Check sheet for the modelled part. Datum: model origin and axes. Units: mm. Face numbers are marked on the shaded views. A direction names the side the tool comes from. Coordinates: 2 decimals unless noted, no trailing zeros. Write each loop counter-clockwise with the first axis right and the second up, starting at its lowest first coordinate (ties: lowest second). Pieces come first, ordered by that corner, then holes. Notation, with made-up numbers: (61.5, 5) - (119.5, 5) arc R17 ccw to (119.5, 12) - close; hole circle Ø9 at (-39, -2). An arc over 180 degrees is marked (long way). Use one line per item in the form item = value. Start each with the question number.
1. Draft check along X on the marked faces 1, 2, 3 and 4. Enter one of: +X half, -X half, draft (parallel to the pull), parting line (faces both ways), or undercut.
2. Scan lines: line 1 along Y through (x, z) = (-7, 67); line 2 along X through (y, z) = (50, 19.5); line 3 along Z through (x, y) = (15, 99). Record each from-to range of solid material in increasing order.
3. Cross-section at C-C on y = -96. Record the boundary of the cut face in (x, z).
4. Tool access check on the marked faces 5, 6 and 7. Record the directions out of +Z, -Z, +X, -X, +Y, -Y that give a thin tool (end or side, any length) a straight path to the whole face; none if there is none.
5. Cross-section at B-B on x = -28.5. Record the boundary of the cut face in (y, z).
6. Cross-section at A-A on z = 11. Record the boundary of the cut face in (x, y).
7. Go/stop test with flat-tipped pins: pin 1 Ø1.8 at (x, z) = (-61.5, -6.5) entering from -Y; pin 2 Ø3 at (x, y) = (-7, -93.5) entering from +Z; pin 3 Ø5 at (x, z) = (12.5, -1) entering from -Y; pin 4 Ø6.5 at (x, z) = (61.5, -6) entering from +Y. Record where each tip stops, or that it passes through.
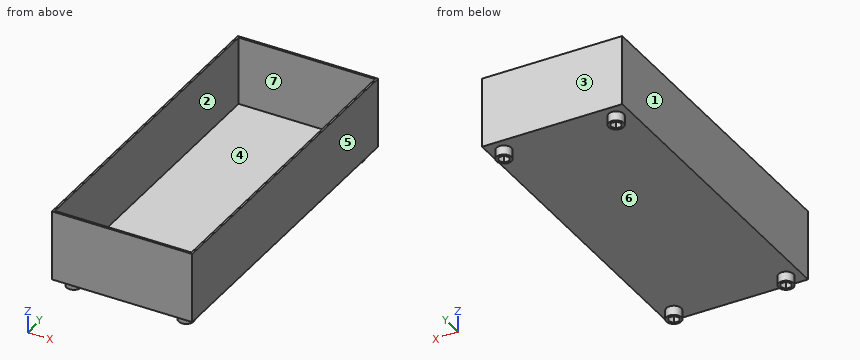
```python
from build123d import *

# Parameters (mm, degrees)
SKETCH1_W           = 150
SKETCH1_H           = 350
BOSS_EXTRUDE1_DEPTH = 75
SHELL1_T            = -2
SKETCH2_R           = 8
BOSS_EXTRUDE2_DEPTH = 10


with BuildPart() as part:
    # Sketch1 → Boss-Extrude1 (new body)
    with BuildSketch(Plane.XY):
        Rectangle(SKETCH1_W, SKETCH1_H)
    extrude(amount=BOSS_EXTRUDE1_DEPTH)

    # Shell1
    shell1_openings = [part.faces().sort_by_distance(p)[0] for p in [
        (0, 0, 75),
    ]]
    offset(amount=SHELL1_T, openings=shell1_openings, kind=Kind.INTERSECTION)

    # Sketch2 → Boss-Extrude2 (add)
    # profile 1 of 4: a face of its own
    with BuildSketch(Plane(origin=(0, 0, 0), x_dir=(-1, 0, 0), z_dir=(0, 0, -1))):
        with Locations((-60, 160)):
            Circle(SKETCH2_R)
        Polygon((-62.973353886, 154.85), (-57.026646114, 154.85), (-54.053292227, 160), (-57.026646114, 165.15), (-62.973353886, 165.15), (-65.946707773, 160), align=None, mode=Mode.SUBTRACT)
    # profile 2 of 4: a face of its own
    with BuildSketch(Plane(origin=(0, 0, 0), x_dir=(-1, 0, 0), z_dir=(0, 0, -1))):
        with Locations(Location((-60, -160, 0), (0, 0, 180))):
            Circle(SKETCH2_R)
        Polygon((-65.946707773, -160), (-62.973353886, -154.85), (-57.026646114, -154.85), (-54.053292227, -160), (-57.026646114, -165.15), (-62.973353886, -165.15), align=None, mode=Mode.SUBTRACT)
    # profile 3 of 4: a face of its own
    with BuildSketch(Plane(origin=(0, 0, 0), x_dir=(-1, 0, 0), z_dir=(0, 0, -1))):
        with Locations((60, -160)):
            Circle(SKETCH2_R)
        Polygon((62.973353886, -165.15), (65.946707773, -160), (62.973353886, -154.85), (57.026646114, -154.85), (54.053292227, -160), (57.026646114, -165.15), align=None, mode=Mode.SUBTRACT)
    # profile 4 of 4: a face of its own
    with BuildSketch(Plane(origin=(0, 0, 0), x_dir=(-1, 0, 0), z_dir=(0, 0, -1))):
        with Locations(Location((60, 160, 0), (0, 0, 180))):
            Circle(SKETCH2_R)
        Polygon((65.946707773, 160), (62.973353886, 154.85), (57.026646114, 154.85), (54.053292227, 160), (57.026646114, 165.15), (62.973353886, 165.15), align=None, mode=Mode.SUBTRACT)
    extrude(amount=BOSS_EXTRUDE2_DEPTH)


solid = part.part
```
Final values:
q1.face_1 = -X half
q1.face_2 = undercut
q1.face_3 = draft
q1.face_4 = undercut
q2.line_1 = -175 to -173, 173 to 175
q2.line_2 = -75 to -73, 73 to 75
q2.line_3 = 0 to 2
q3.outline = (-75, 0) - (75, 0) - (75, 75) - (73, 75) - (73, 2) - (-73, 2) - (-73, 75) - (-75, 75) - close
q4.face_5 = +Z, -Z, +X, +Y, -Y
q4.face_6 = -Z
q4.face_7 = +Z
q5.outline = (-175, 0) - (175, 0) - (175, 75) - (173, 75) - (173, 2) - (-173, 2) - (-173, 75) - (-175, 75) - close
q6.outline = (-75, -175) - (75, -175) - (75, 175) - (-75, 175) - close; hole (-73, -173) - (73, -173) - (73, 173) - (-73, 173) - close
q7.pin_1 = -167.98
q7.pin_2 = 2
q7.pin_3 = -175
q7.pin_4 = 168
